Could you check a few things on this model? Use its own coordinates, in mm. Round coordinates to 2 decimals unless told otherwise and drop trailing zeros. Loops run counter-clockwise (first coordinate to the right, second up) from the corner with the lowest first, then second, coordinate; pieces in that order, holes last. Notation, with made-up numbers: (75.25, -6.5) -> (113.25, -6.5) arc R11 ccw to (113.25, 7.5) -> close; hole circle Ø6 at (75, 32.5). An arc over 180 degrees is marked (long way). One line per item, written item: value.
```python
from build123d import *

# Parameters (mm, degrees)
EXTRUDE_1_DEPTH = 12


with BuildPart() as part:
    # 草图1 → 凸台-拉伸1 (new body)
    with BuildSketch(Plane(origin=(0, 0, 0), x_dir=(1, 0, 0), z_dir=(0, 1, 0))):
        Polygon((0, 0), (130, 0), (130, 150), (60, 150), (60, 180), (10, 180), (10, 150), (0, 150), align=None)
    extrude(amount=EXTRUDE_1_DEPTH)


solid = part.part
```
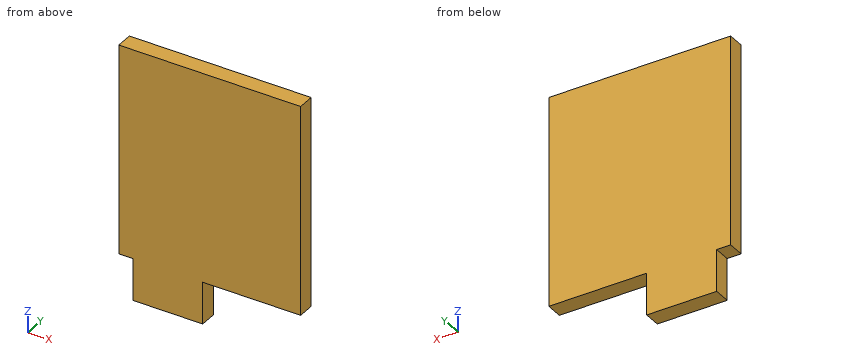
(1) Imagine slicing it at B-B on x = 105. Write out the boundary of the cut face in (y, z).
Results below:
outline: (0, -150) -> (12, -150) -> (12, 0) -> (0, 0) -> close
(2) Please list where these lines run through material, in increasing order: L1, parallel to X at y = 5.5, z = -161.5; L2, parallel to Z at x = 100, y = 6.
Results below:
L1: x = 10 to 60
L2: z = -150 to 0
(3) For pin 1 Ø5 at (x, y) = (81.5, 9.5) entering from -Z; pin 2 Ø3.5 at (y, z) = (9, -170.5) entering from +X; pin 3 Ø6 at (y, z) = (4, -171.5) entering from -X, each with a flat end and sliding along its axis, tell me the tip position at first contact or that it passes through.
Results below:
pin 1: stops at z = -150
pin 2: stops at x = 60
pin 3: stops at x = 10
(4) Imagine slicing it at A-A on y = 4. Write out the boundary of the cut face in (x, z), then the cut area to 3 significant figures.
Results below:
outline: (0, -150) -> (10, -150) -> (10, -180) -> (60, -180) -> (60, -150) -> (130, -150) -> (130, 0) -> (0, 0) -> close
area: 21,000 mm²
